Work out the finished part from the listing and answer in its coordinate system (mm). A direction names the side the tool comes from. Coordinates: 2 decimals unless noted, no trailing zeros. Order: outer loops, then holes, each group sorted by start corner. A loop starts at its lowest first (then second) coordinate and runs counter-clockwise, first axis right, second up. Notation, with made-up numbers: (13, 19) -> (21, 19) arc R27 cw to (21, 41) -> close; hole circle Ø5 at (-30.75, 75.5). An arc over 180 degrees is marked (long way). Write item = value, one per line. Start each with the question number.
Q1. Which of the six approach directions +Z, -Z, +X, -X, +Y, -Y give full straight-line access (tool end or side, diameter ignored) to faces 1 (the flat face through (-5, 0, -28)), 2 (the flat face through (193.469, 14.79, 62.386)), 3 (the cylindrical face through (1.302, 6.409, -111.415))?
Q2. The part is cut by section D-D, the plane x = -322.5. Determine the outline of the cut face in (y, z).
Q3. The part is cut by section B-B, the plane z = -11.5. Determine the outline of the cut face in (x, y), plus the area to 3 significant figures.
Q4. For a pull along X with two mould halves and no side action, classify faces 4 (the flat face through (381.5, 15, 7)), 5 (the flat face through (-7, 13, -99)), 6 (the flat face through (-367, 15, 116.5)), 7 (the cylindrical face through (-4.975, 21.619, -106.062)) as +X half, -X half, draft (parallel to the pull), parting line (faces both ways), or undercut.
Q5. Flat-ended cylindrical pins translate along their axes: pin 1 (12 mm diameter, centred on x = 0, z = -101.5, fed in from +Y); pin 2 (8 mm diameter, centred on x = -181, y = 15, fed in from +Z); pin 3 (6 mm diameter, centred on x = -50.21, y = 15, fed in from -Z); pin 4 (6 mm diameter, centred on y = 15, z = 101.5, fed in from +X). Find the tip coordinate at first contact, or state that the pin passes through.
Q6. Straight lines are drawn through the part: L1, parallel to Z at x = 0, y = 3.5; L2, parallel to Z at x = -370, y = 15; L3, parallel to X at y = 26.25, z = -56.5. For each, find the intervals that lie inside material, in ascending order. Write a range as from..to.
Q7. The part is cut by section C-C, the plane y = 4.5. Determine the outline of the cut face in (x, z), plus the area to 3 significant figures.
Q8. The part is cut by section A-A, the plane x = 0. Determine the outline of the cut face in (y, z), plus the area to 3 significant figures.
```python
from build123d import *

# Parameters (mm, degrees)
SKETCH_1_W                = 763
SKETCH_1_H                = 233
EXTRUDE_1_DEPTH           = 30
CHAMFER_1_SIZE            = 10
CUT_EXTRUDE_1_DEPTH       = 401.018124589
CUT_EXTRUDE_1_DEPTH_BACK  = 30
FILLET_1_R                = 60
HOLE_WIZARD_1_D           = 13.5
HOLE_WIZARD_1_CBORE_D     = 20
HOLE_WIZARD_1_CBORE_DEPTH = 13
HOLE_WIZARD_M12_1_D       = 10.2
HOLE_WIZARD_M12_1_DEPTH   = 29.25
HOLE_WIZARD_M12_1_TIP     = 3.064389157
HOLE_WIZARD_M12_2_D       = 10.2
HOLE_WIZARD_M12_2_DEPTH   = 29.25
HOLE_WIZARD_M12_2_TIP     = 3.064389157
HOLE_WIZARD_M12_3_D       = 10.2
HOLE_WIZARD_M12_3_DEPTH   = 29.25
HOLE_WIZARD_M12_3_TIP     = 3.064389157


with BuildPart() as part:
    # 草图1 → 凸台-拉伸1 (new body)
    with BuildSketch(Plane(origin=(0, 0, 0), x_dir=(1, 0, 0), z_dir=(0, 1, 0))):
        Rectangle(SKETCH_1_W, SKETCH_1_H)
    extrude(amount=EXTRUDE_1_DEPTH)

    # 倒角1
    chamfer_1_edges = [part.edges().sort_by_distance(p)[0] for p in [
        (-381.5, 15, -116.5),
        (381.5, 15, -116.5),
    ]]
    chamfer(chamfer_1_edges, length=CHAMFER_1_SIZE)

    # 草图2 → 切除-拉伸1 (cut, two sides: drawn at the far end of the back side and taken through both)
    with BuildSketch(Plane(origin=(0, 30, 0), x_dir=(1, 0, 0), z_dir=(0, 1, 0)).offset(-CUT_EXTRUDE_1_DEPTH_BACK)):
        Polygon((-1816.285660926, -618.078120257), (-351.5, -116.5), (-21.5, -3.5), (21.5, -3.5), (351.5, -116.5), (1816.285660926, -618.078120257), (1816.285660926, -3714.642437803), (-1816.285660926, -3714.642437803), align=None)
    extrude(amount=CUT_EXTRUDE_1_DEPTH + CUT_EXTRUDE_1_DEPTH_BACK, mode=Mode.SUBTRACT)

    # 圆角1
    fillet_1_edges = [part.edges().sort_by_distance(p)[0] for p in [
        (21.5, 15, 3.5),
        (-21.5, 15, 3.5),
    ]]
    fillet(fillet_1_edges, radius=FILLET_1_R)

    # 打孔尺寸(%根据)内六角圆柱头螺钉的类型1 (through all)
    with Locations(Plane(origin=(0, 0, 0), x_dir=(-1, 0, 0), z_dir=(0, -1, 0))):
        with Locations((0, 11.5), (0, 56.5), (0, 101.5)):
            CounterBoreHole(HOLE_WIZARD_1_D / 2, HOLE_WIZARD_1_CBORE_D / 2, HOLE_WIZARD_1_CBORE_DEPTH)

    # M12 螺纹孔1
    with Locations(Plane(origin=(0, 0, -116.5), x_dir=(-1, 0, 0), z_dir=(0, 0, -1))):
        with Locations((351.5, 15), (251.071428571, 15), (150.642857143, 15), (50.214285714, 15), (-50.214285714, 15), (-150.642857143, 15), (-251.071428571, 15), (-351.5, 15)):
            Hole(HOLE_WIZARD_M12_1_D / 2, depth=HOLE_WIZARD_M12_1_DEPTH)
            with Locations((0, 0, -(HOLE_WIZARD_M12_1_DEPTH + HOLE_WIZARD_M12_1_TIP / 2))):  # 118° drill point
                Cone(0, HOLE_WIZARD_M12_1_D / 2, HOLE_WIZARD_M12_1_TIP, mode=Mode.SUBTRACT)

    # M12 螺纹孔2
    with Locations(Plane.ZY.offset(381.5)):
        with Locations((-76.5, 15), (12.5, 15), (101.5, 15)):
            Hole(HOLE_WIZARD_M12_2_D / 2, depth=HOLE_WIZARD_M12_2_DEPTH)
            with Locations((0, 0, -(HOLE_WIZARD_M12_2_DEPTH + HOLE_WIZARD_M12_2_TIP / 2))):  # 118° drill point
                Cone(0, HOLE_WIZARD_M12_2_D / 2, HOLE_WIZARD_M12_2_TIP, mode=Mode.SUBTRACT)

    # M12 螺纹孔3
    with Locations(Plane(origin=(381.5, 0, 0), x_dir=(0, 0, -1), z_dir=(1, 0, 0))):
        with Locations((76.5, 15), (-12.5, 15), (-101.5, 15)):
            Hole(HOLE_WIZARD_M12_3_D / 2, depth=HOLE_WIZARD_M12_3_DEPTH)
            with Locations((0, 0, -(HOLE_WIZARD_M12_3_DEPTH + HOLE_WIZARD_M12_3_TIP / 2))):  # 118° drill point
                Cone(0, HOLE_WIZARD_M12_3_D / 2, HOLE_WIZARD_M12_3_TIP, mode=Mode.SUBTRACT)


solid = part.part
```
Model answer:
q1.face_1 = +Z, -Z, +X, -X, -Y
q1.face_2 = +Z, +Y, -Y
q1.face_3 = -Y
q2.outline = (0, -116.5) -> (30, -116.5) -> (30, 106.57) -> (0, 106.57) -> close
q3.outline = (-381.5, 0) -> (-10, 0) -> (-10, 13) -> (-6.75, 13) -> (-6.75, 30) -> (-381.5, 30) -> close; (6.75, 13) -> (10, 13) -> (10, 0) -> (381.5, 0) -> (381.5, 30) -> (6.75, 30) -> close
q3.area = 22,400 mm2
q4.face_4 = +X half
q4.face_5 = undercut
q4.face_6 = draft
q4.face_7 = undercut
q5.pin_1 = through
q5.pin_2 = 59.49
q5.pin_3 = -85.99
q5.pin_4 = 350.99
q6.L1 = -116.5..-111.5, -91.5..-66.5, -46.5..-21.5, -1.5..3.5
q6.L2 = -116.5..-81.6, -71.4..7.4, 17.6..96.4, 106.6..116.5
q6.L3 = -381.5..-6.75, 6.75..381.5
q7.outline = (-381.5, -106.5) -> (-371.5, -116.5) -> (371.5, -116.5) -> (381.5, -106.5) -> (381.5, 116.5) -> (351.5, 116.5) -> (30.95, 6.74) arc R60 cw to (11.51, 3.5) -> (-11.51, 3.5) arc R60 cw to (-30.95, 6.74) -> (-351.5, 116.5) -> (-381.5, 116.5) -> close; hole circle Ø20 at (0, -101.5); hole circle Ø20 at (0, -56.5); hole circle Ø20 at (0, -11.5)
q7.area = 135,000 mm2
q8.outline = (0, -116.5) -> (30, -116.5) -> (30, -108.25) -> (13, -108.25) -> (13, -111.5) -> (0, -111.5) -> close; (0, -91.5) -> (13, -91.5) -> (13, -94.75) -> (30, -94.75) -> (30, -63.25) -> (13, -63.25) -> (13, -66.5) -> (0, -66.5) -> close; (0, -46.5) -> (13, -46.5) -> (13, -49.75) -> (30, -49.75) -> (30, -18.25) -> (13, -18.25) -> (13, -21.5) -> (0, -21.5) -> close; (0, -1.5) -> (13, -1.5) -> (13, -4.75) -> (30, -4.75) -> (30, 3.5) -> (0, 3.5) -> close
q8.area = 2,130 mm2
